```python
from build123d import *

# Parameters (mm, degrees)
BOSS_EXTRUDE1_DEPTH = 167


with BuildPart() as part:
    # Sketch1 → Boss-Extrude1 (new body)
    with BuildSketch(Plane.XY):
        with BuildLine():
            Line((0, 0), (30, 0))
            Line((30, 0), (30, 1))
            ThreePointArc((30, 1), (29.414213562, 2.414213562), (28, 3))
            Line((28, 3), (5, 3))
            ThreePointArc((5, 3), (3.585786438, 3.585786438), (3, 5))
            Line((3, 5), (3, 28))
            ThreePointArc((3, 28), (2.414213562, 29.414213562), (1, 30))
            Line((1, 30), (0, 30))
            Line((0, 30), (0, 0))
        make_face()
    extrude(amount=BOSS_EXTRUDE1_DEPTH)


solid = part.part
```
Source: CAD feature listing. Evaluate the final solid. Frame: model axes, mm. A direction names the side the tool comes from. Coordinates: 2 decimals unless noted, no trailing zeros. Loops run counter-clockwise (first coordinate to the right, second up) from the corner with the lowest first, then second, coordinate; pieces in that order, holes last. Notation, with made-up numbers: (53, 38) -> (69, 38) arc R7 ccw to (69, 51) -> close; hole circle Ø6 at (-19, 39). An arc over 180 degrees is marked (long way). One line per item, written item: value. Start each with the question number.
Q1. Section query B-B, the plane x = 22. Return the cut outline in (y, z).
Q2. Section query A-A, the plane z = 14. Return the cut outline in (x, y), and give its area (3 significant figures).
Q3. Contact query for flat-ended pins moving along their axis: P1, Ø8, axis at y = 8, z = 24, coming from the +X side; P2, Ø5, axis at x = 8, z = 79.5, coming from the +Y side; P3, Ø1.5, axis at y = 11.5, z = 145, coming from the +X side; P4, Ø4, axis at y = 14, z = 149, coming from the -X side. Output: stop coordinate, or through.
Q4. Line query: line 1 along Y through (x, z) = (18.25, 46.5); line 2 along X through (y, z) = (1.5, 157). Output: solid intervals per line, ascending.
Q5. Set-up query: faces 1 (the face through (17, 3, 82)), 2 (the face through (15, 0, 82)). Return all of +Z, -Z, +X, -X, +Y, -Y with unobstructed straight access to the full face (end or side cutting, diameter ignored); none if empty.
Results:
1. outline: (0, 0) -> (3, 0) -> (3, 167) -> (0, 167) -> close
2. outline: (0, 0) -> (30, 0) -> (30, 1) arc R2 ccw to (28, 3) -> (5, 3) arc R2 cw to (3, 5) -> (3, 28) arc R2 ccw to (1, 30) -> (0, 30) -> close
2. area: 170 mm^2
3. P1: x = 3.27
3. P2: y = 3
3. P3: x = 3
3. P4: x = 0
4. line 1: 0 to 3
4. line 2: 0 to 29.94
5. face 1: +Z, -Z, +X, +Y
5. face 2: +Z, -Z, +X, -X, -Y
